from build123d import *

# Parameters (mm, degrees)
SKETCH1_W             = 120
SKETCH1_H             = 100
BOSS_EXTRUDE1_DEPTH   = 10
M8_TAPPED_HOLE1_D     = 6.8
M8_TAPPED_HOLE1_DEPTH = 19.75
M8_TAPPED_HOLE1_TIP   = 2.042926105


with BuildPart() as part:
    # Sketch1 → Boss-Extrude1 (new body)
    with BuildSketch(Plane.XY):
        Rectangle(SKETCH1_W, SKETCH1_H)
    extrude(amount=BOSS_EXTRUDE1_DEPTH)

    # M8 Tapped Hole1
    with Locations(Plane.XY.offset(10)):
        with Locations((45, -35), (-45, -35), (-45, 35), (45, 35)):
            Hole(M8_TAPPED_HOLE1_D / 2, depth=M8_TAPPED_HOLE1_DEPTH)
            with Locations((0, 0, -(M8_TAPPED_HOLE1_DEPTH + M8_TAPPED_HOLE1_TIP / 2))):  # 118° drill point
                Cone(0, M8_TAPPED_HOLE1_D / 2, M8_TAPPED_HOLE1_TIP, mode=Mode.SUBTRACT)


solid = part.part
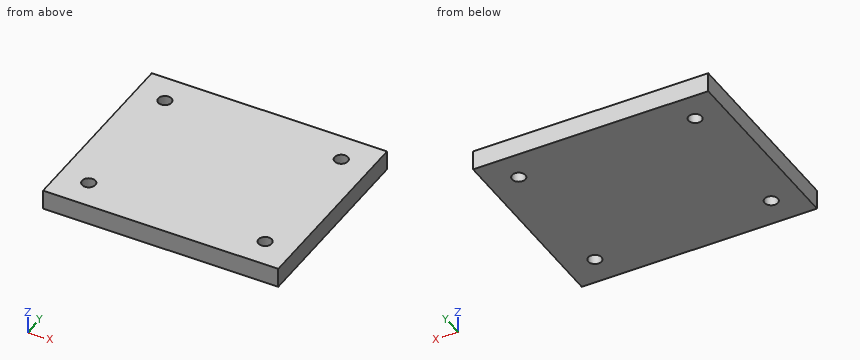
The model under review builds one solid part; all positions refer to its coordinate system, in mm. Coordinates: 2 decimals unless noted, no trailing zeros. Order: outer loops, then holes, each group sorted by start corner. A loop starts at its lowest first (then second) coordinate and runs counter-clockwise, first axis right, second up. Notation, with made-up numbers: (54.5, 1) -> (72.5, 1) arc R33 cw to (72.5, 34) -> close; hole circle Ø8 at (53, 45). An arc over 180 degrees is marked (long way). Answer in a Markdown table with one row per item.
(1) Consider section A-A (x = 45). Write out the cut boundary in (y, z), plus the area to 3 significant figures.
Answers:
| item | result |
|---|---|
| outline | (-50, 0) -> (-38.4, 0) -> (-38.4, 10) -> (-50, 10) -> close; (-31.6, 0) -> (31.6, 0) -> (31.6, 10) -> (-31.6, 10) -> close; (38.4, 0) -> (50, 0) -> (50, 10) -> (38.4, 10) -> close |
| area | 864 mm² |
(2) Wall thickness on line 1 along Y through (x, z) = (45, 6); line 2 along Y through (x, z) = (-44, 2.25): over which ranges is each line inside the solid? List them lowest first.
Answers:
| item | result |
|---|---|
| line 1 | -50 to -38.4, -31.6 to 31.6, 38.4 to 50 |
| line 2 | -50 to -38.25, -31.75 to 31.75, 38.25 to 50 |
(3) Insertion check: pin 1 (4 mm diameter, centred on x = 45, y = 35, fed in from +Z). The pin has a flat end and moves straight along its axis. Give the tip position at first contact, or say it passes through.
Answers:
| item | result |
|---|---|
| pin 1 | through |
(4) Consider section B-B (y = -35). Write out the cut boundary in (x, z), plus the area to 3 significant figures.
Answers:
| item | result |
|---|---|
| outline | (-60, 0) -> (-48.4, 0) -> (-48.4, 10) -> (-60, 10) -> close; (-41.6, 0) -> (41.6, 0) -> (41.6, 10) -> (-41.6, 10) -> close; (48.4, 0) -> (60, 0) -> (60, 10) -> (48.4, 10) -> close |
| area | 1,060 mm² |
